Can you work these out from the drawing? Everything is in mm from the part's minimum corner. Coordinates: 2 decimals unless noted, no trailing zeros. Loops run counter-clockwise (first coordinate to the right, second up) from the corner with the lowest first, then second, coordinate; pieces in that order, holes last. Notation, with made-up numbers: M -13,-3.5 L 17,-3.5 A22 cw 17,10.5 Z; hole C 45,-28 d4. An arc over 180 degrees is marked long. Write each question's results on one line, items separated by ' | '.
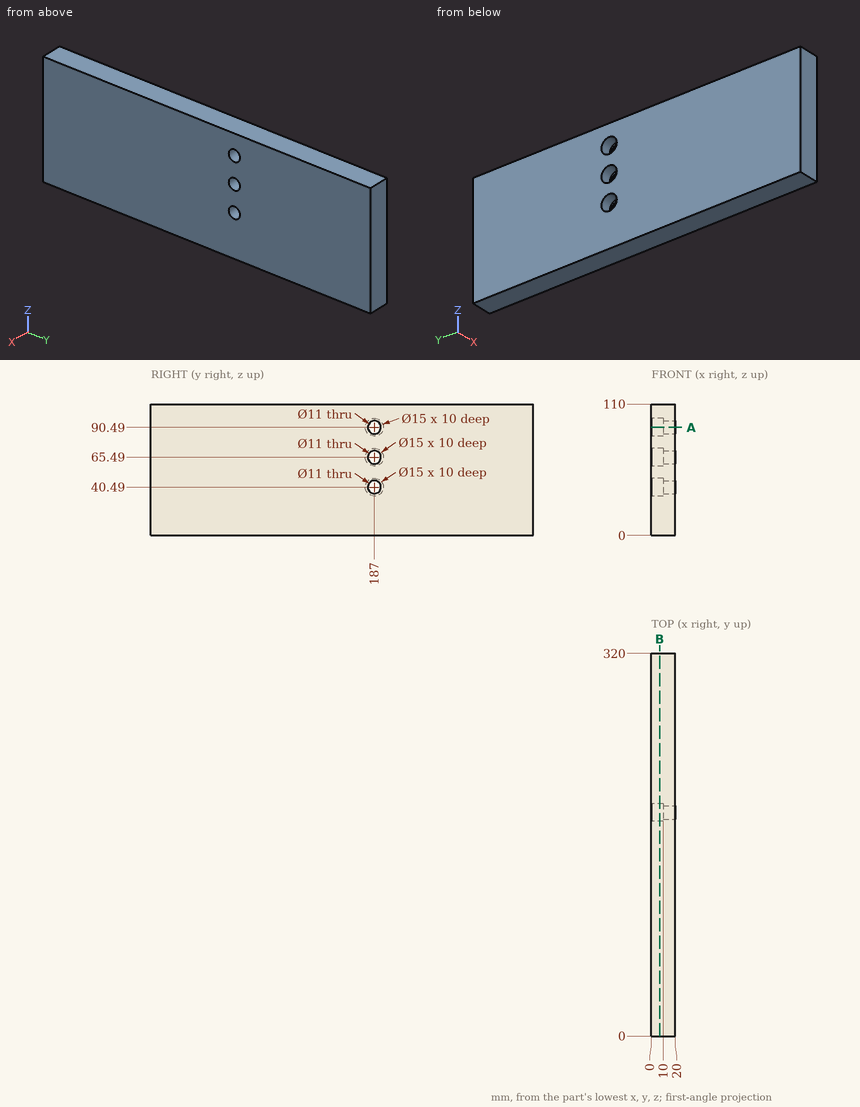
(1) Please list where these lines run through material, in increasing order: probe 1 along Y at (x, z) = (5.5, 65.49); probe 2 along Y at (x, z) = (15, 65.49). Write a range as from..to.
Reported:
probe 1: y = 0..179.5, 194.5..320 | probe 2: y = 0..181.5, 192.5..320
(2) Imagine slicing it at A-A, the plane z = 90.49. List the corners of the cut face in (x, y) for me.
Reported:
outline: M 0,0 L 20,0 L 20,181.5 L 10,181.5 L 10,179.5 L 0,179.5 Z; M 0,194.5 L 10,194.5 L 10,192.5 L 20,192.5 L 20,320 L 0,320 Z
(3) Will these pins go through, and if not, where does the flat tip stop? P1, Ø13.5, axis at y = 187, z = 40.49, coming from the -X side; P2, Ø6.5, axis at y = 187, z = 65.49, coming from the +X side; P3, Ø12, axis at y = 187, z = 93.5, coming from the -X side.
Reported:
P1: stops at x = 10 | P2: passes through | P3: stops at x = 0
(4) Imagine slicing it at B-B, the plane x = 7. List the corners of the cut face in (y, z) for me.
Reported:
outline: M 0,0 L 320,0 L 320,110 L 0,110 Z; hole C 187,40.49 d15; hole C 187,65.49 d15; hole C 187,90.49 d15
